from build123d import *

# Parameters (mm, degrees)
SKETCH1_W                                           = 92
SKETCH1_H                                           = 120
BOSS_EXTRUDE1_DEPTH                                 = 5
SKETCH2_R                                           = 11
CUT_EXTRUDE1_DEPTH                                  = 77.26270386
M4_TAPPED_HOLE1_D                                   = 3.3
CBORE_FOR_M4_HEX_SOCKET_HEAD_CAP_SCREW1_D           = 4.5
CBORE_FOR_M4_HEX_SOCKET_HEAD_CAP_SCREW1_CBORE_D     = 8
CBORE_FOR_M4_HEX_SOCKET_HEAD_CAP_SCREW1_CBORE_DEPTH = 4.4
CBORE_FOR_M5_HEX_SOCKET_HEAD_CAP_SCREW1_D           = 5.5
CBORE_FOR_M5_HEX_SOCKET_HEAD_CAP_SCREW1_DEPTH       = 10.1
CBORE_FOR_M5_HEX_SOCKET_HEAD_CAP_SCREW1_CBORE_D     = 10
CBORE_FOR_M5_HEX_SOCKET_HEAD_CAP_SCREW1_CBORE_DEPTH = 5.4
CBORE_FOR_M5_HEX_SOCKET_HEAD_CAP_SCREW1_TIP         = 1.652366702


with BuildPart() as part:
    # Sketch1 → Boss-Extrude1 (new, symmetric)
    with BuildSketch(Plane(origin=(0, 0, 0), x_dir=(0, 0, -1), z_dir=(1, 0, 0))):
        Rectangle(SKETCH1_W, SKETCH1_H)
    extrude(amount=BOSS_EXTRUDE1_DEPTH, both=True)

    # Sketch2 → Cut-Extrude1 (cut, through all)
    with BuildSketch(Plane(origin=(5, 0, 0), x_dir=(0, 0, -1), z_dir=(1, 0, 0))):
        with Locations((0, 30)):
            Circle(SKETCH2_R)
    extrude(amount=-CUT_EXTRUDE1_DEPTH, mode=Mode.SUBTRACT)

    # M4 Tapped Hole1 (through all)
    with Locations(Plane(origin=(5, 0, 0), x_dir=(0, 0, -1), z_dir=(1, 0, 0))):
        with Locations((-41, -30), (-41, -18), (41, -30), (41, -18)):
            Hole(M4_TAPPED_HOLE1_D / 2)

    # CBORE for M4 Hex Socket Head Cap Screw1 (through all)
    with Locations(Plane.ZY.offset(5)):
        with Locations((-41, 51), (-41, 30), (-41, 9), (41, 51), (41, 30), (41, 9)):
            CounterBoreHole(CBORE_FOR_M4_HEX_SOCKET_HEAD_CAP_SCREW1_D / 2, CBORE_FOR_M4_HEX_SOCKET_HEAD_CAP_SCREW1_CBORE_D / 2, CBORE_FOR_M4_HEX_SOCKET_HEAD_CAP_SCREW1_CBORE_DEPTH)

    # CBORE for M5 Hex Socket Head Cap Screw1
    with Locations(Plane.ZY.offset(5)):
        with Locations((-14, 48), (14, 48), (-14, 12), (14, 12)):
            CounterBoreHole(CBORE_FOR_M5_HEX_SOCKET_HEAD_CAP_SCREW1_D / 2, CBORE_FOR_M5_HEX_SOCKET_HEAD_CAP_SCREW1_CBORE_D / 2, CBORE_FOR_M5_HEX_SOCKET_HEAD_CAP_SCREW1_CBORE_DEPTH, depth=CBORE_FOR_M5_HEX_SOCKET_HEAD_CAP_SCREW1_DEPTH)
            with Locations((0, 0, -(CBORE_FOR_M5_HEX_SOCKET_HEAD_CAP_SCREW1_DEPTH + CBORE_FOR_M5_HEX_SOCKET_HEAD_CAP_SCREW1_TIP / 2))):  # 118° drill point
                Cone(0, CBORE_FOR_M5_HEX_SOCKET_HEAD_CAP_SCREW1_D / 2, CBORE_FOR_M5_HEX_SOCKET_HEAD_CAP_SCREW1_TIP, mode=Mode.SUBTRACT)


solid = part.part
Design review of the part built by this model. Coordinates are the model's own, in mm. A direction names the side the tool comes from. Coordinates: 2 decimals unless noted, no trailing zeros. Order: outer loops, then holes, each group sorted by start corner. A loop starts at its lowest first (then second) coordinate and runs counter-clockwise, first axis right, second up. Notation, with made-up numbers: M 77,52.25 L 96,52.25 A21 cw 96,90.25 Z; hole C 50,-29 d8. An arc over 180 degrees is marked long. Use a Markdown table: item, result.
(1) Add section A-A (z = 14). Give the boundary of the cut face in (x, y), then the cut area to 3 significant figures.
Worked answers:
| item | result |
|---|---|
| outline | M -5,-60 L 5,-60 L 5,9.25 L 0.4,9.25 L 0.4,7 L -5,7 Z; M -5,17 L 0.4,17 L 0.4,14.75 L 5,14.75 L 5,45.25 L 0.4,45.25 L 0.4,43 L -5,43 Z; M -5,53 L 0.4,53 L 0.4,50.75 L 5,50.75 L 5,60 L -5,60 Z |
| area | 1,040 mm2 |
(2) For faces 1 (the flat face through (0.4, 45.8, -11.8)), 2 (the cylindrical face through (2.239, 30.099, -38.752)), list the 3-axis set-ups (+Z, -Z, +X, -X, +Y, -Y) from which the entire face can be reached by the end or side of a thin tool; tool diameter is ignored.
Worked answers:
| item | result |
|---|---|
| face 1 | -X |
| face 2 | +X, -X |
(3) Wall thickness on probe 1 along Y at (x, z) = (2.75, -14); probe 2 along Y at (x, z) = (-1.2, 14); probe 3 along Y at (x, z) = (-2, -41): over which ranges is each line inside the solid? List them lowest first.
Worked answers:
| item | result |
|---|---|
| probe 1 | y = -60 to 9.25, 14.75 to 45.25, 50.75 to 60 |
| probe 2 | y = -60 to 7, 17 to 43, 53 to 60 |
| probe 3 | y = -60 to -31.65, -28.35 to -19.65, -16.35 to 5, 13 to 26, 34 to 47, 55 to 60 |
(4) Add section D-D (z = 0.5). Give the boundary of the cut face in (x, y), then the cut area to 3 significant figures.
Worked answers:
| item | result |
|---|---|
| outline | M -5,-60 L 5,-60 L 5,19.01 L -5,19.01 Z; M -5,40.99 L 5,40.99 L 5,60 L -5,60 Z |
| area | 980 mm2 |
(5) For P1, Ø4, axis at y = 51, z = 42.5, coming from the -X side, flat-tipped, find the tip position at first contact; note if it passes through.
Worked answers:
| item | result |
|---|---|
| P1 | stops at x = -0.6 |
(6) Add section B-B (y = 30). Give the boundary of the cut face in (x, z).
Worked answers:
| item | result |
|---|---|
| outline | M -5,-46 L 5,-46 L 5,-43.25 L -0.6,-43.25 L -0.6,-45 L -5,-45 Z; M -5,-37 L -0.6,-37 L -0.6,-38.75 L 5,-38.75 L 5,-11 L -5,-11 Z; M -5,11 L 5,11 L 5,38.75 L -0.6,38.75 L -0.6,37 L -5,37 Z; M -5,45 L -0.6,45 L -0.6,43.25 L 5,43.25 L 5,46 L -5,46 Z |
(7) Draft analysis for pull direction Y (two halves, no side actions). For faces 3 (the cylindrical face through (-2.831, 33.966, -41.521)), 4 (the flat face through (5, 1, 1)), 5 (the flat face through (-0.6, 28, -39)), 6 (the flat face through (0, 60, 1)), state which applies: released by +Y, released by -Y, zero draft, split by the parting line, or undercut.
Worked answers:
| item | result |
|---|---|
| face 3 | undercut |
| face 4 | zero draft |
| face 5 | undercut |
| face 6 | released by +Y |
(8) Add section C-C (x = 3.75). Count the separate pieces of the cut face and the enclosed holes in it, then the cut area to 3 significant figures.
Worked answers:
| item | result |
|---|---|
| separate pieces | 1 |
| enclosed holes | 15 |
| area | 10,400 mm2 |
